```python
from build123d import *

# Parameters (mm, degrees)
SKETCH1_R               = 4
BOSS_EXTRUDE1_DEPTH     = 60
SKETCH2_R               = 7.5
BOSS_EXTRUDE2_DEPTH     = 4
CUT_EXTRUDE1_DEPTH      = 61.930288035
CUT_EXTRUDE1_DEPTH_BACK = 61.930288035
SKETCH3_R               = 1.35
CHAMFER1_SIZE           = 0.5


with BuildPart() as part:
    # Sketch1 → Boss-Extrude1 (new body)
    with BuildSketch(Plane.XY):
        Circle(SKETCH1_R)
    extrude(amount=BOSS_EXTRUDE1_DEPTH)

    # Sketch2 → Boss-Extrude2 (add)
    with BuildSketch(Plane(origin=(0, 0, 0), x_dir=(-1, 0, 0), z_dir=(0, 0, -1))):
        Circle(SKETCH2_R)
    extrude(amount=BOSS_EXTRUDE2_DEPTH)

    # Sketch3 → Cut-Extrude1 (cut, two sides: drawn at the far end of the back side and taken through both)
    with BuildSketch(Plane(origin=(0, 0, 0), x_dir=(1, 0, 0), z_dir=(0, 1, 0)).offset(-CUT_EXTRUDE1_DEPTH_BACK)):
        with Locations(Location((0, -56, 0), (0, 0, 270))):
            Circle(SKETCH3_R)
    extrude(amount=CUT_EXTRUDE1_DEPTH + CUT_EXTRUDE1_DEPTH_BACK, mode=Mode.SUBTRACT)

    # Chamfer1
    chamfer1_edges = [part.edges().sort_by_distance(p)[0] for p in [
        (-4, 0, 60),
        (7.5, 0, 0),
        (7.5, 0, -4),
    ]]
    chamfer(chamfer1_edges, length=CHAMFER1_SIZE)


solid = part.part
```
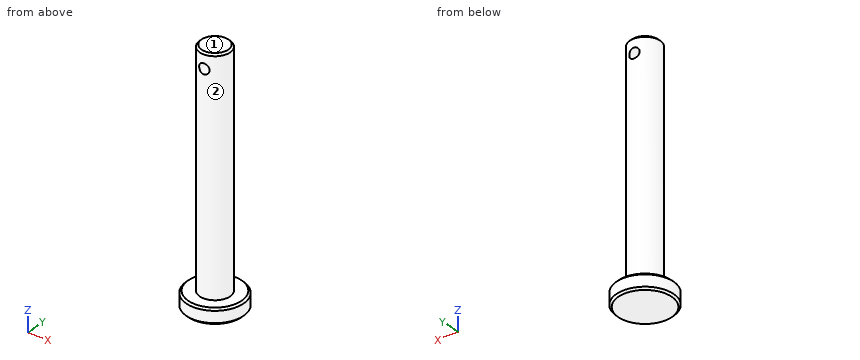
Geometry: final body of the model. Coordinates: model frame, mm. Face numbers are marked on the shaded views. A direction names the side the tool comes from. Round coordinates to 2 decimals unless told otherwise and drop trailing zeros. Loops run counter-clockwise (first coordinate to the right, second up) from the corner with the lowest first, then second, coordinate; pieces in that order, holes last. Notation, with made-up numbers: (-24, -32) -> (-14, -32) arc R7 cw to (-14, -26) -> close; hole circle Ø11 at (61.25, 45). An arc over 180 degrees is marked (long way). Use one line per item in the form item = value. Start each with the question number.
1) First-contact query: P1, Ø3, axis at x = -4, z = 17, coming from the -Y side; P2, Ø8, axis at y = -3.5, z = 5.5, coming from the +X side; P3, Ø5, axis at x = 6, z = 31.5, coming from the -Y side. Flat tips, straight axial feed; report the tip coordinate or a pass-through.
2) Access query for the marked faces 1 and 2. Directions: +Z, -Z, +X, -X, +Y, -Y. A direction counts if a zero-diameter tool reaches every point of the face in a straight line with its end or side. Return the directions, or none.
3) Section B-B on y = 0. Output: boundary loops of the cut face in (x, z), then the cut area to 3 significant figures.
4) Section C-C on z = 56. Output: boundary loops of the cut face in (x, y).
5) Section A-A on x = 0. Output: boundary loops of the cut face in (y, z).
6) Line query: L1, parallel to Z at x = 0, y = -2; L2, parallel to Z at x = 6, y = -0.25; L3, parallel to Y at x = 0.25, z = 17. Output: solid intervals per line, ascending.
Response:
q1.P1 = -3.12
q1.P2 = 4
q1.P3 = -1.94
q2.face_1 = +Z, +X, -X, +Y, -Y
q2.face_2 = +Z
q3.outline = (-7.5, -3.5) -> (-7, -4) -> (7, -4) -> (7.5, -3.5) -> (7.5, -0.5) -> (7, 0) -> (4, 0) -> (4, 59.5) -> (3.5, 60) -> (-3.5, 60) -> (-4, 59.5) -> (-4, 0) -> (-7, 0) -> (-7.5, -0.5) -> close; hole circle Ø2.7 at (0, 56)
q3.area = 534 mm^2
q4.outline = (-1.35, -3.77) -> (-1.35, 3.77) arc R4 ccw to start; (1.35, -3.77) arc R4 ccw to (1.35, 3.77) -> close
q5.outline = (-7.5, -3.5) -> (-7, -4) -> (7, -4) -> (7.5, -3.5) -> (7.5, -0.5) -> (7, 0) -> (4, 0) -> (4, 54.65) -> (-4, 54.65) -> (-4, 0) -> (-7, 0) -> (-7.5, -0.5) -> close; (-4, 57.35) -> (4, 57.35) -> (4, 59.5) -> (3.5, 60) -> (-3.5, 60) -> (-4, 59.5) -> close
q6.L1 = -4 to 54.65, 57.35 to 60
q6.L2 = -4 to 0
q6.L3 = -3.99 to 3.99
